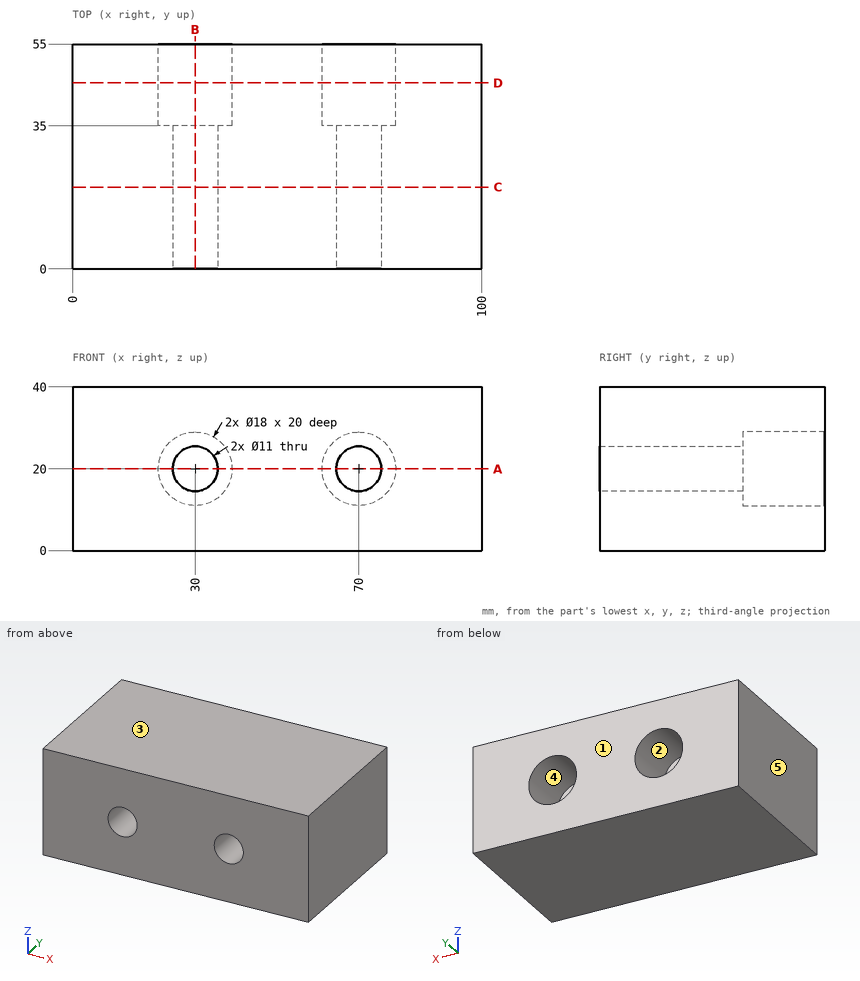
Part print with two shaded views. Sizes in mm from the minimum x, y, z corner. A direction names the side the tool comes from. Round coordinates to 2 decimals unless told otherwise and drop trailing zeros. Order: outer loops, then holes, each group sorted by start corner. A loop starts at its lowest first (then second) coordinate and runs counter-clockwise, first axis right, second up. Notation, with made-up numbers: (9.5, 23.5) - (39.5, 23.5) arc R32 ccw to (39.5, 58.5) - close; hole circle Ø5 at (-26, 6.25). An arc over 180 degrees is marked (long way). Answer in a Markdown table with one row per item. Add a question column.
(1) Mould opens along X. For the marked faces 3, 4 and 5 say: +X half, -X half, draft (parallel to the pull), parting line (faces both ways), or undercut.
(2) Probe L1, parallel to X at y = 27.5, z = 20; L2, parallel to X at y = 46.5, z = 20; L3, parallel to Z at x = 70, y = 12. List the from-to ranges inside material, lowest first. Write a range as [from, to].
(3) 3-axis set-ups, long thin cutter, end or side, ignore diameter. For the marked faces 1 and 2: which of +Z, -Z, +X, -X, +Y, -Y reach the whole face in a straight line?
(4) Band-saw the part on A-A on z = 20. List the corners of the cut face in (x, y), and give its area (3 significant figures).
(5) Band-saw the part on D-D on y = 45.5. List the corners of the cut face in (x, z).
(6) Band-saw the part on B-B on x = 30. List the corners of the cut face in (y, z).
(7) Band-saw the part on C-C on y = 20. List the corners of the cut face in (x, z).
(8) Drop a flat-ended pin along its axis: pin 1 Ø12.5 at (x, z) = (30, 20) entering from +Y. Give the stop position or say it passes through.
Data:
| question | item | result |
|---|---|---|
| 1 | face 3 | draft |
| 1 | face 4 | undercut |
| 1 | face 5 | -X half |
| 2 | L1 | x = [0, 24.5], [35.5, 64.5], [75.5, 100] |
| 2 | L2 | x = [0, 21], [39, 61], [79, 100] |
| 2 | L3 | z = [0, 14.5], [25.5, 40] |
| 3 | face 1 | +Z, -Z, +X, -X, +Y |
| 3 | face 2 | +Y |
| 4 | outline | (0, 0) - (24.5, 0) - (24.5, 35) - (21, 35) - (21, 55) - (0, 55) - close; (35.5, 0) - (64.5, 0) - (64.5, 35) - (61, 35) - (61, 55) - (39, 55) - (39, 35) - (35.5, 35) - close; (75.5, 0) - (100, 0) - (100, 55) - (79, 55) - (79, 35) - (75.5, 35) - close |
| 4 | area | 4,010 mm^2 |
| 5 | outline | (0, 0) - (100, 0) - (100, 40) - (0, 40) - close; hole circle Ø18 at (30, 20); hole circle Ø18 at (70, 20) |
| 6 | outline | (0, 0) - (55, 0) - (55, 11) - (35, 11) - (35, 14.5) - (0, 14.5) - close; (0, 25.5) - (35, 25.5) - (35, 29) - (55, 29) - (55, 40) - (0, 40) - close |
| 7 | outline | (0, 0) - (100, 0) - (100, 40) - (0, 40) - close; hole circle Ø11 at (30, 20); hole circle Ø11 at (70, 20) |
| 8 | pin 1 | stops at y = 35 |
